Source: three-view drawing plus pictorial views. Frame: mm from the lowest corner of the part. Give positions to 0.01 mm unless a question says otherwise; leave off trailing zeros. Loops run counter-clockwise (first coordinate to the right, second up) from the corner with the lowest first, then second, coordinate; pieces in that order, holes last. Notation, with made-up numbers: (-37.75, 27) - (3.25, 27) arc R10 ccw to (3.25, 31) - close; hole circle Ø2 at (11.5, 41.5). An arc over 180 degrees is marked (long way). Answer as a JSON object with one key per item and string values. Group by question number.
(1) Material intervals for L1, parallel to Y at x = 54.5, z = 5.75; L2, parallel to X at y = 139.5, z = 1.75; L3, parallel to X at y = 118.5, z = 2, sorted ascending.
(2) Section query A-A (z = 8.25). Return loops of the section in (x, y).
(3) Section query C-C (y = 31). Return loops of the section in (x, z).
(4) Section query B-B (y = 57). Return loops of the section in (x, z).
(5) Pin query (flat end, axial travel): P1, Ø6, axis at x = 39, z = 6.5, coming from the -Y side; P2, Ø5, axis at x = 61, z = 2.5, coming from the -Y side; P3, Ø6, axis at y = 129, z = 2.5, coming from the -X side. Return the tip coordinate at first contact, or that it passes through.
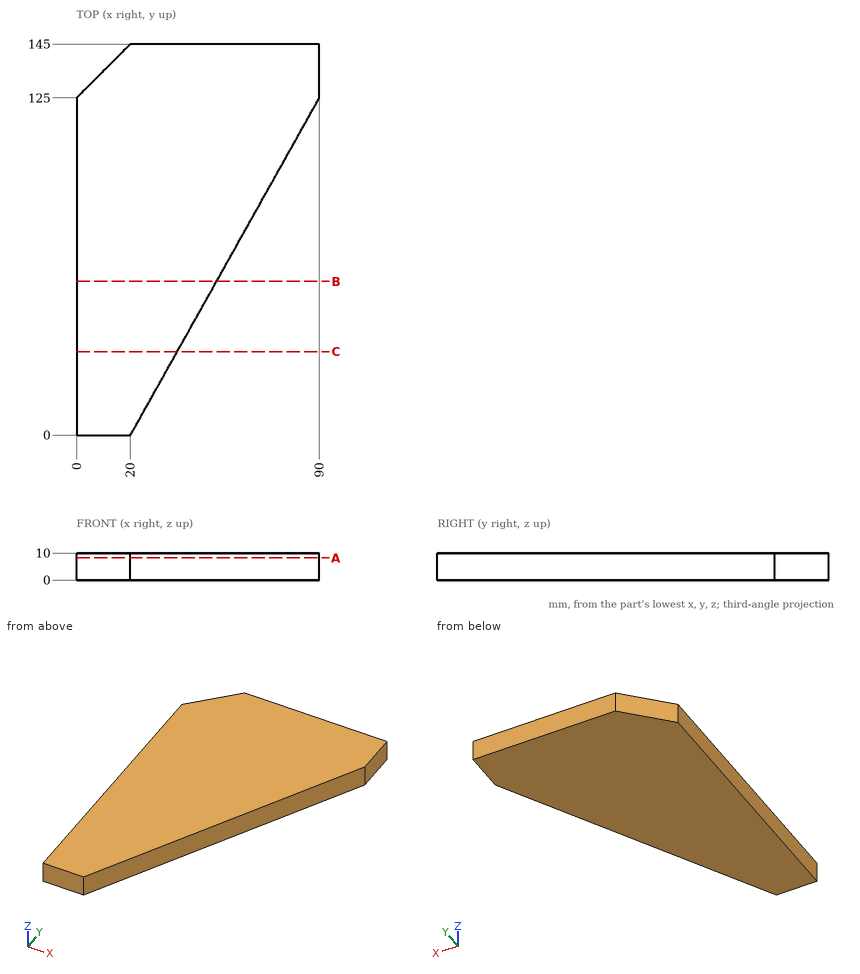
Recorded:
{
 "1": {"L1": "y = 61.61 to 145", "L2": "x = 14.5 to 90", "L3": "x = 0 to 86.36"},
 "2": {"outline": "(0, 0) - (20, 0) - (90, 125) - (90, 145) - (20, 145) - (0, 125) - close"},
 "3": {"outline": "(0, 0) - (37.36, 0) - (37.36, 10) - (0, 10) - close"},
 "4": {"outline": "(0, 0) - (51.92, 0) - (51.92, 10) - (0, 10) - close"},
 "5": {"P1": "stops at y = 28.57", "P2": "stops at y = 68.75", "P3": "stops at x = 1"}
}
